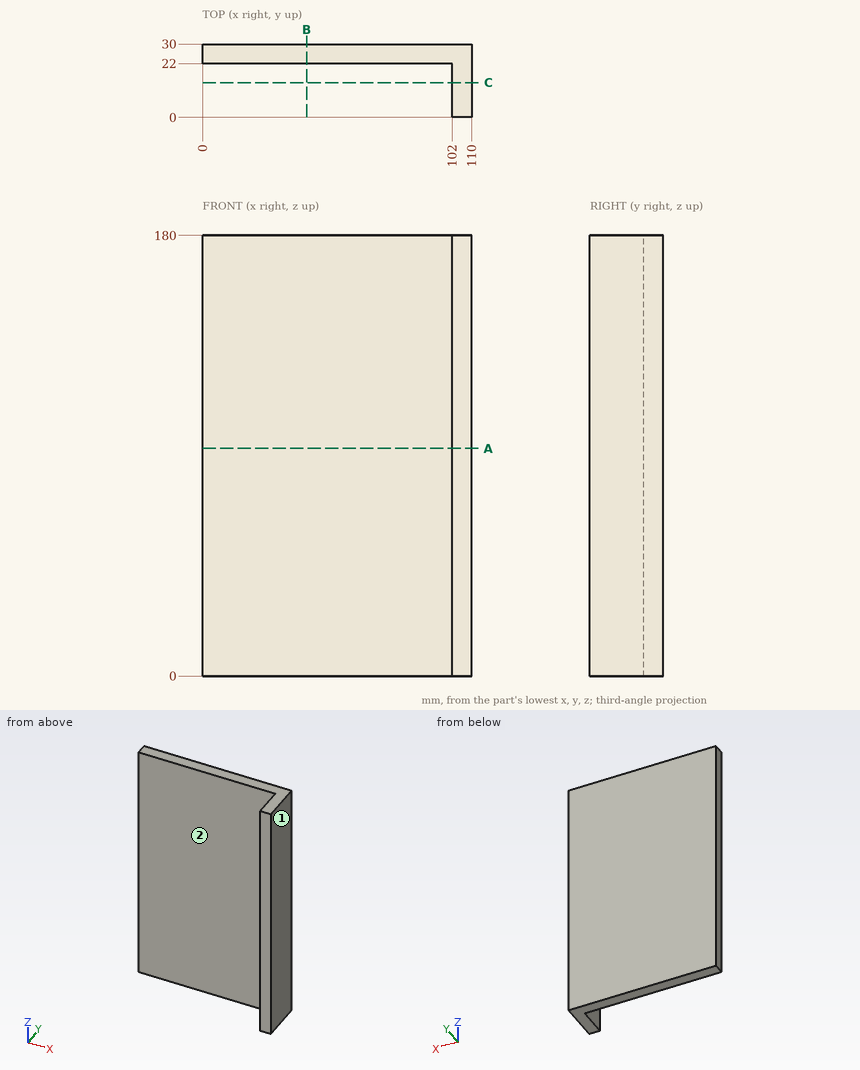
For this review, use the dimensioned drawing (mm, ordinates from the lowest corner) and the shaded views. A direction names the side the tool comes from. Coordinates: 2 decimals unless noted, no trailing zeros. Write each loop counter-clockwise with the first axis right and the second up, starting at its lowest first coordinate (ties: lowest second). Pieces come first, ordered by that corner, then holes. Notation, with made-up numbers: (72, -30.5) -> (131, -30.5) arc R25 cw to (131, -13.5) -> close; hole circle Ø1 at (56, 57.25). An arc over 180 degrees is marked (long way). Write each question's results on one line, items separated by ' | '. Start each with the question number.
(1) Take a section at B-B on x = 42.5. Write out the cut boundary in (y, z), and give its area (3 significant figures).
(2) Clearance check with a flat-ended pin moving along its axis: P1, Ø3, axis at y = 14.5, z = 100, coming from the -X side. State where the tip first meets the part, or that it passes through.
(3) Take a section at A-A on z = 93. Write out the cut boundary in (x, y), and give its area (3 significant figures).
(4) For line 1 along Y through (x, z) = (41, 57.5); line 2 along X through (y, z) = (13, 113), list the stretches that pass through material, from the lowest coordinate up. Write a range as from..to.
(5) Tool access review of the marked faces 1 and 2: name each direction out of +Z, -Z, +X, -X, +Y, -Y from which nothing blocks a thin tool from reaching the whole face with its end or side.
(6) Take a section at C-C on y = 14.25. Write out the cut boundary in (x, z), and give its area (3 significant figures).
Results found:
1) outline: (22, 0) -> (30, 0) -> (30, 180) -> (22, 180) -> close | area: 1,440 mm2
2) P1: stops at x = 102
3) outline: (0, 22) -> (102, 22) -> (102, 0) -> (110, 0) -> (110, 30) -> (0, 30) -> close | area: 1,060 mm2
4) line 1: y = 22..30 | line 2: x = 102..110
5) face 1: +Z, -Z, +X, +Y, -Y | face 2: +Z, -Z, -X, -Y
6) outline: (102, 0) -> (110, 0) -> (110, 180) -> (102, 180) -> close | area: 1,440 mm2
